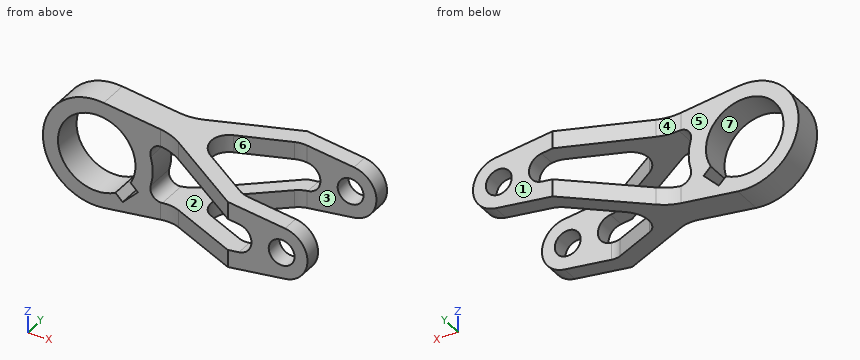
```python
from build123d import *

# Parameters (mm, degrees)
LEVER_BLANK_DEPTH             = 30
HUB_BORE_36_WITH_KEYWAY_DEPTH = 100.247166206
HOLE_12_SKETCH_R              = 6
HOLE_12_DEPTH                 = 100.247166206
RELIEF_SLOT_DEPTH             = 100.247166206
FORK_OUTLINE_CUT_DEPTH        = 30
ARM_LIGHTENING_WINDOWS_DEPTH  = 30


with BuildPart() as part:
    # Side Profile Sketch → Lever Blank (new, symmetric)
    with BuildSketch(Plane(origin=(0, 0, 0), x_dir=(1, 0, 0), z_dir=(0, 1, 0))):
        with BuildLine():
            Line((-46.75, 24.787849846), (51.56, 11.898167926))
            ThreePointArc((51.56, 11.898167926), (62, 0), (51.56, -11.898167926))
            Line((51.56, -11.898167926), (-46.75, -24.787849846))
            ThreePointArc((-46.75, -24.787849846), (-75, 0), (-46.75, 24.787849846))
        make_face()
    extrude(amount=LEVER_BLANK_DEPTH, both=True)

    # Hub Bore Sketch → Hub Bore Ø36 with Keyway (cut, through all)
    with BuildSketch(Plane(origin=(0, 30, 0), x_dir=(1, 0, 0), z_dir=(0, 1, 0))):
        with BuildLine():
            Line((-41.308514645, 15.762553167), (-37.97918472, 19.091883092))
            Line((-37.97918472, 19.091883092), (-30.908116908, 12.02081528))
            Line((-30.908116908, 12.02081528), (-34.237446833, 8.691485355))
            ThreePointArc((-34.237446833, 8.691485355), (-62.727922061, -12.727922061), (-41.308514645, 15.762553167))
        make_face()
    extrude(amount=-HUB_BORE_36_WITH_KEYWAY_DEPTH, mode=Mode.SUBTRACT)

    # Hole Ø12 Sketch → Hole Ø12 (cut, through all)
    with BuildSketch(Plane(origin=(0, 30, 0), x_dir=(1, 0, 0), z_dir=(0, 1, 0))):
        with Locations(Location((50, 0, 0), (0, 0, 270))):
            Circle(HOLE_12_SKETCH_R)
    extrude(amount=-HOLE_12_DEPTH, mode=Mode.SUBTRACT)

    # Relief Slot Sketch → Relief Slot (cut, through all)
    with BuildSketch(Plane(origin=(0, 30, 0), x_dir=(1, 0, 0), z_dir=(0, 1, 0))):
        with BuildLine():
            Line((-19.488879252, 13.145103734), (30.18, 6.632886717))
            ThreePointArc((30.18, 6.632886717), (36, 0), (30.18, -6.632886717))
            Line((30.18, -6.632886717), (-19.488879252, -13.145103734))
            ThreePointArc((-19.488879252, -13.145103734), (-23.922952707, -11.455681264), (-24.949066043, -6.822944804))
            ThreePointArc((-24.949066043, -6.822944804), (-24, 0), (-24.949066043, 6.822944804))
            ThreePointArc((-24.949066043, 6.822944804), (-23.922952707, 11.455681264), (-19.488879252, 13.145103734))
        make_face()
    extrude(amount=-RELIEF_SLOT_DEPTH, mode=Mode.SUBTRACT)

    # Fork Outline Sketch → Fork Outline Cut (cut, symmetric)
    with BuildSketch(Plane.XY):
        with BuildLine():
            Line((-75, 30), (-75, 7))
            Line((-75, 7), (-20.340076505, 7))
            ThreePointArc((-20.340076505, 7), (-15.180741335, 7.676924142), (-10.370654019, 9.661873939))
            Line((-10.370654019, 9.661873939), (25, 30))
            Line((25, 30), (-75, 30))
        make_face()
        with BuildLine():
            Line((-75, -30), (-75, -7))
            Line((-75, -7), (-20.340076505, -7))
            ThreePointArc((-20.340076505, -7), (-15.180741335, -7.676924142), (-10.370654019, -9.661873939))
            Line((-10.370654019, -9.661873939), (25, -30))
            Line((25, -30), (-75, -30))
        make_face()
    extrude(amount=FORK_OUTLINE_CUT_DEPTH, both=True, mode=Mode.SUBTRACT)

    # Arm Windows Sketch → Arm Lightening Windows (cut, symmetric)
    with BuildSketch(Plane.XY):
        with BuildLine():
            Line((62, 22), (29.806068854, 22))
            ThreePointArc((29.806068854, 22), (27.226401269, 21.661537929), (24.821357612, 20.669063031))
            Line((24.821357612, 20.669063031), (3.951792394, 8.669063031))
            ThreePointArc((3.951792394, 8.669063031), (-1.063496363, 0), (3.951792394, -8.669063031))
            Line((3.951792394, -8.669063031), (24.821357612, -20.669063031))
            ThreePointArc((24.821357612, -20.669063031), (27.226401269, -21.661537929), (29.806068854, -22))
            Line((29.806068854, -22), (62, -22))
            Line((62, -22), (62, 22))
        make_face()
    extrude(amount=ARM_LIGHTENING_WINDOWS_DEPTH, both=True, mode=Mode.SUBTRACT)


solid = part.part
```
Read the model definition and answer for the solid it produces. Units are mm, in the model's axes. Face numbers are marked on the shaded views. A direction names the side the tool comes from. Round coordinates to 2 decimals unless told otherwise and drop trailing zeros. Write each loop counter-clockwise with the first axis right and the second up, starting at its lowest first coordinate (ties: lowest second). Pieces come first, ordered by that corner, then holes. Notation, with made-up numbers: M 78,3.5 L 112,3.5 A7 ccw 112,10.5 Z; hole C 40,11.5 d9. An arc over 180 degrees is marked long. One line per item, written item: value.
Q1. Straight lines are drawn through the part: line 1 (Y direction, x = 39.5, z = -4); line 2 (X direction, y = -1, z = 0); line 3 (X direction, y = -26, z = 0). For each, find the intervals that lie inside material, in ascending order. Write a range as [from, to].
Data:
line 1: [-30, -22], [22, 30]
line 2: [-75, -68], [-32, -24]
line 3: [36, 44], [56, 62]
Q2. Find section C-C on y = 5.5. Write down the section's boundary in (x, z).
Data:
outline: M -46.75,-24.79 L 0.58,-18.58 L 0.58,-10.51 L -19.49,-13.15 A5 cw -24.95,-6.82 A25 ccw -24.95,6.82 A5 cw -19.49,13.15 L 0.58,10.51 L 0.58,18.58 L -46.75,24.79 A25 ccw long Z; hole M -41.31,-15.76 L -37.98,-19.09 L -30.91,-12.02 L -34.24,-8.69 A18 ccw long Z
Q3. Find section D-D on x = 50. Write down the section's boundary in (y, z).
Data:
outline: M -30,-12.1 L -22,-12.1 L -22,-6 L -30,-6 Z; M -30,6 L -22,6 L -22,12.1 L -30,12.1 Z; M 22,-12.1 L 30,-12.1 L 30,-6 L 22,-6 Z; M 22,6 L 30,6 L 30,12.1 L 22,12.1 Z
Q4. Find section A-A on z = 0. Write down the section's boundary in (x, y), plus the area to 3 significant figures.
Data:
outline: M -75,-7 L -68,-7 L -68,7 L -75,7 Z; M -32,-7 L -24,-7 L -24,7 L -32,7 Z; M 36,-30 L 44,-30 L 44,-22 L 36,-22 Z; M 36,22 L 44,22 L 44,30 L 36,30 Z; M 56,-30 L 62,-30 L 62,-22 L 56,-22 Z; M 56,22 L 62,22 L 62,30 L 56,30 Z
area: 434 mm2
Q5. Flat-ended cylindrical pins translate along their axes: pin 1 Ø25 at (x, z) = (-56.5, -6.5) entering from +Y; pin 2 Ø23.5 at (x, z) = (48, -3) entering from +Y; pin 3 Ø8 at (x, y) = (17, 23) entering from -Z; pin 4 Ø12 at (y, z) = (17, -10) entering from +X. Find the tip coordinate at first contact, or state that the pin passes through.
Data:
pin 1: y = 7
pin 2: y = 30
pin 3: z = -16.95
pin 4: x = 59.97
Q6. For a pull along X with two mould halves and no side action, classify the marked faces 4, 5, 6 and 7 as +X half, -X half, draft (parallel to the pull), parting line (faces both ways), or undercut.
Data:
face 4: -X half
face 5: draft
face 6: +X half
face 7: undercut
Q7. Find section B-B on x = -50. Write down the section's boundary in (y, z).
Data:
outline: M -7,-25 L 7,-25 L 7,-18 L -7,-18 Z; M -7,18 L 7,18 L 7,25 L -7,25 Z
Q8. Which of the six approach directions +Z, -Z, +X, -X, +Y, -Y give full straight-line access (tool end or side, diameter ignored) to the marked faces 1, 2 and 3?
Data:
face 1: +Z, -Z, +X, -X, +Y
face 2: +Y, -Y
face 3: +Z, -Z, +X
